Model file for the job. Use its own axes, mm. Coordinates: 2 decimals unless noted, no trailing zeros. Order: outer loops, then holes, each group sorted by start corner. A loop starts at its lowest first (then second) coordinate and runs counter-clockwise, first axis right, second up.
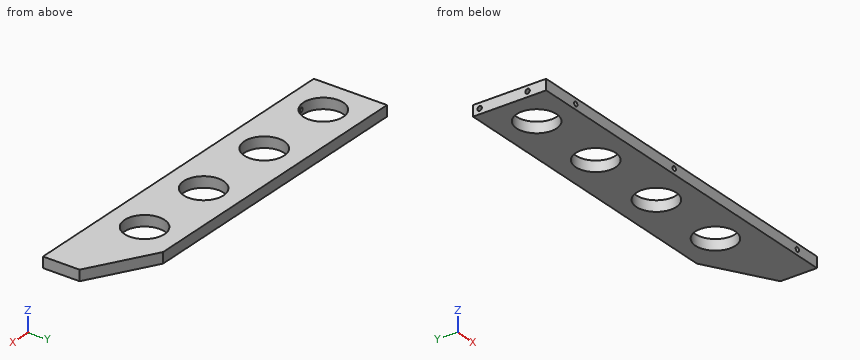
from build123d import *

# Parameters (mm, degrees)
SKETCH_1_W               = 550
SKETCH_1_H               = 110
EXTRUDE_1_DEPTH          = 8
CUT_EXTRUDE_4_DEPTH      = 281.902118184
CUT_EXTRUDE_4_DEPTH_BACK = 281.902118184
HOLE1_D                  = 6.75
HOLE1_DEPTH              = 26
HOLE1_TIP                = 2.027904589
HOLE11_D                 = 6.75
HOLE11_DEPTH             = 28
HOLE11_TIP               = 2.027904589
SKETCH_10_R              = 30
CUT_EXTRUDE_5_DEPTH      = 281.902118184


with BuildPart() as part:
    # 草图1 → 凸台-拉伸1 (new, symmetric)
    with BuildSketch(Plane.XY):
        Rectangle(SKETCH_1_W, SKETCH_1_H)
    extrude(amount=EXTRUDE_1_DEPTH, both=True)

    # 草图9 → 切除-拉伸4 (cut, two sides: drawn at the far end of the back side and taken through both)
    with BuildSketch(Plane.XY.offset(8).offset(-CUT_EXTRUDE_4_DEPTH_BACK)):
        Polygon((-786.302283658, 612.743159162), (179.737205584, 55), (275, 0), (1241.039489242, -557.743159162), (2356.525807565, 1374.335819322), (329.184034665, 2544.822137646), align=None)
    extrude(amount=CUT_EXTRUDE_4_DEPTH + CUT_EXTRUDE_4_DEPTH_BACK, mode=Mode.SUBTRACT)

    # Hole1
    with Locations(Plane(origin=(-134.213455343, -55, 9.167765698), x_dir=(1, 0, 0), z_dir=(0, -1, 0))):
        with Locations((-80.786544657, -9.167765698), (119.213455343, -9.167765698), (369.213455343, -9.167765698)):
            Hole(HOLE1_D / 2, depth=HOLE1_DEPTH)
            with Locations((0, 0, -(HOLE1_DEPTH + HOLE1_TIP / 2))):  # 118° drill point
                Cone(0, HOLE1_D / 2, HOLE1_TIP, mode=Mode.SUBTRACT)

    # Hole11
    with Locations(Plane(origin=(-275, -17.832234302, -14.213455343), x_dir=(0, 0, 1), z_dir=(-1, 0, 0))):
        with Locations((14.213455343, -9.167765698), (14.213455343, 62.832234302)):
            Hole(HOLE11_D / 2, depth=HOLE11_DEPTH)
            with Locations((0, 0, -(HOLE11_DEPTH + HOLE11_TIP / 2))):  # 118° drill point
                Cone(0, HOLE11_D / 2, HOLE11_TIP, mode=Mode.SUBTRACT)

    # 草图10 → 切除-拉伸5 (cut, through all)
    with BuildSketch(Plane.XY.offset(8)):
        with Locations((-220, 0)):
            Circle(SKETCH_10_R)
        with Locations((-100, 0)):
            Circle(SKETCH_10_R)
        with Locations(Location((23.038475773, 0, 0), (0, 0, 180))):
            Circle(SKETCH_10_R)
        with Locations(Location((143.038475773, 0, 0), (0, 0, 180))):
            Circle(SKETCH_10_R)
    extrude(amount=-CUT_EXTRUDE_5_DEPTH, mode=Mode.SUBTRACT)


solid = part.part
Q1. Drop flat-ended pins along their axis: P1, Ø5, axis at y = 5.5, z = 4, coming from the +X side; P2, Ø8, axis at y = 45, z = 0, coming from the -X side; P3, Ø4, axis at x = -215, z = 0, coming from the -Y side. Give the stop position or say it passes through.
Established:
P1: stops at x = 269.8
P2: stops at x = -275
P3: stops at y = 29.17
Q2. Cut at D-D, the plane x = 190. List the corners of the cut face in (y, z).
Established:
outline: (-55, -8) - (49.07, -8) - (49.07, 8) - (-55, 8) - close
Q3. Cut at A-A, the plane x = -100. List the corners of the cut face in (y, z), plus the area to 3 significant figures.
Established:
outline: (-55, -8) - (-30, -8) - (-30, 8) - (-55, 8) - close; (30, -8) - (55, -8) - (55, 8) - (30, 8) - close
area: 800 mm2
Q4. Cut at B-B, the plane y = -8. List the corners of the cut face in (x, z).
Established:
outline: (-275, -8) - (-248.91, -8) - (-248.91, 8) - (-275, 8) - close; (-191.09, -8) - (-128.91, -8) - (-128.91, 8) - (-191.09, 8) - close; (-71.09, -8) - (-5.88, -8) - (-5.88, 8) - (-71.09, 8) - close; (51.95, -8) - (114.12, -8) - (114.12, 8) - (51.95, 8) - close; (171.95, -8) - (275, -8) - (275, 8) - (171.95, 8) - close
Q5. Probe line 1 (Y direction, x = -258.5, z = 0) (3 decimals); line 2 (Z direction, x = 235, y = -42.25) (3 decimals); line 3 (X direction, y = -9.5, z = -2). List the from-to ranges inside material, lowest first.
Established:
line 1: y = -55 to -30.375, -23.625 to 41.625, 48.375 to 55
line 2: z = -8 to -3.375, 3.375 to 8
line 3: x = -275 to -248.46, -191.54 to -128.46, -71.54 to -5.42, 51.49 to 114.58, 171.49 to 275
Q6. Cut at C-C, the plane y = 18.5. List the corners of the cut face in (x, z).
Established:
outline: (-275, -8) - (-243.62, -8) - (-243.62, 8) - (-275, 8) - close; (-196.38, -8) - (-123.62, -8) - (-123.62, 8) - (-196.38, 8) - close; (-76.38, -8) - (-0.58, -8) - (-0.58, 8) - (-76.38, 8) - close; (46.66, -8) - (119.42, -8) - (119.42, 8) - (46.66, 8) - close; (166.66, -8) - (242.96, -8) - (242.96, 8) - (166.66, 8) - close
